Design review of the part shown in the three views and the two pictorial views. Dimensions are in mm from the part's minimum x, y and z. Round coordinates to 2 decimals unless told otherwise and drop trailing zeros. Order: outer loops, then holes, each group sorted by start corner. A loop starts at its lowest first (then second) coordinate and runs counter-clockwise, first axis right, second up. Notation, with made-up numbers: (38.25, 4.5) - (42.25, 4.5) arc R33 ccw to (42.25, 36.5) - close; hole circle Ø8 at (-0.75, 5.5). An arc over 180 degrees is marked (long way). Use CSV: the item, a comma, the result in double quotes.
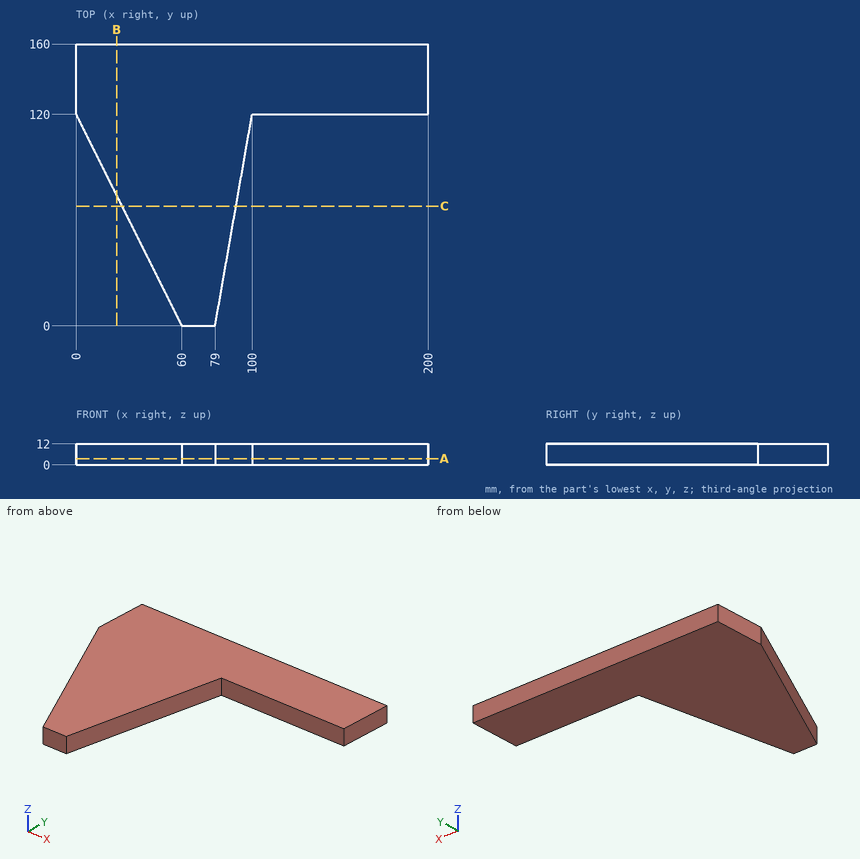
1) To check wall thickness, follow L1, parallel to Y at x = 156, z = 1.75; L2, parallel to X at y = 63.5, z = 2; L3, parallel to X at y = 57, z = 9 (3 decimals). State the ranges of each line that lie inside material, in increasing order. Write a range as from..to.
Data:
L1,"y = 120..160"
L2,"x = 28.25..90.11"
L3,"x = 31.5..88.975"
2) We need section B-B (x = 23). Give the boundary of the cut face in (y, z), then the cut area to 3 significant figures.
Data:
outline,"(74, 0) - (160, 0) - (160, 12) - (74, 12) - close"
area,"1,030 mm2"
3) We need section C-C (y = 68). Give the boundary of the cut face in (x, z), then the cut area to 3 significant figures.
Data:
outline,"(26, 0) - (90.9, 0) - (90.9, 12) - (26, 12) - close"
area,"779 mm2"
4) We need section A-A (z = 3.5). Give the boundary of the cut face in (x, y), then the cut area to 3 significant figures.
Data:
outline,"(0, 120) - (60, 0) - (79, 0) - (100, 120) - (200, 120) - (200, 160) - (0, 160) - close"
area,"15,100 mm2"
5) Insertion check: pin 1 Ø5 at (y, z) = (47.5, 4) entering from +X; pin 2 Ø6 at (x, z) = (158.5, 7.5) entering from -Y; pin 3 Ø6 at (y, z) = (110, 11) entering from +X (3 decimals). Each pin has a flat end and moves straight along its axis. Give the tip position at first contact, or say it passes through.
Data:
pin 1,"stops at x = 87.75"
pin 2,"stops at y = 120"
pin 3,"stops at x = 98.775"
